```python
from build123d import *

# Parameters (mm, degrees)
SKETCH_1_R          = 62.5
SKETCH_1_R_2        = 45
EXTRUDE_1_DEPTH     = 18
CUT_EXTRUDE_1_DEPTH = 18


with BuildPart() as part:
    # 草图1 → 凸台-拉伸1 (new body)
    with BuildSketch(Plane.XY):
        Circle(SKETCH_1_R)
        Circle(SKETCH_1_R_2, mode=Mode.SUBTRACT)
    extrude(amount=EXTRUDE_1_DEPTH)

    # 草图2 → 切除-旋转1 (revolve, cut)
    with BuildSketch(Plane(origin=(0, 0, 0), x_dir=(1, 0, 0), z_dir=(0, 1, 0)), mode=Mode.PRIVATE) as cut_revolve_1_sk:
        Polygon((62.5, -4), (62.5, 0), (56, 0), align=None)
        Polygon((62.5, -14), (62.5, -18), (56, -18), align=None)
    revolve(cut_revolve_1_sk.sketch.rotate(Axis((0, 0, -32.669833972), (0, 0, 1)), 180), axis=Axis((0, 0, -32.669833972), (0, 0, 1)), mode=Mode.SUBTRACT)

    # 草图3 → 切除-拉伸1 (cut)
    with BuildSketch(Plane(origin=(0, 0, 0), x_dir=(-1, 0, 0), z_dir=(0, 0, -1))):
        with BuildLine():
            Line((-6, 62.211333373), (-6, 57.211333373))
            Line((-6, 57.211333373), (6, 57.211333373))
            Line((6, 57.211333373), (6, 62.211333373))
            ThreePointArc((6, 62.211333373), (0, 62.5), (-6, 62.211333373))
        make_face()
        with BuildLine():
            Line((62.211333373, 6), (57.211333373, 6))
            Line((57.211333373, 6), (57.211333373, -6))
            Line((57.211333373, -6), (62.211333373, -6))
            ThreePointArc((62.211333373, -6), (62.5, 0), (62.211333373, 6))
        make_face()
        with BuildLine():
            Line((6, -62.211333373), (6, -57.211333373))
            Line((6, -57.211333373), (-6, -57.211333373))
            Line((-6, -57.211333373), (-6, -62.211333373))
            ThreePointArc((-6, -62.211333373), (0, -62.5), (6, -62.211333373))
        make_face()
        with BuildLine():
            Line((-62.211333373, -6), (-57.211333373, -6))
            Line((-57.211333373, -6), (-57.211333373, 6))
            Line((-57.211333373, 6), (-62.211333373, 6))
            ThreePointArc((-62.211333373, 6), (-62.5, 0), (-62.211333373, -6))
        make_face()
    extrude(amount=-CUT_EXTRUDE_1_DEPTH, mode=Mode.SUBTRACT)


solid = part.part
```
Can you work these out from the model? Positions are in its coordinate system, mm. A direction names the side the tool comes from. Round coordinates to 2 decimals unless told otherwise and drop trailing zeros. Loops run counter-clockwise (first coordinate to the right, second up) from the corner with the lowest first, then second, coordinate; pieces in that order, holes last. Notation, with made-up numbers: M -8,12.5 L 9,12.5 A35 ccw 9,45.5 Z; hole C 35,37.5 d7. An arc over 180 degrees is marked long. Answer as a JSON object with one key per item and string values. Group by question number.
Q1. We'd pull the mould along Y, two halves only. Please class faces 5 (the flat face through (-57.211, 0, 9)), 6 (the flat face through (60, -6, 9)), 7 (the cylindrical face through (-44.619, -43.766, 8.93)), 8 (the flat face through (6, 60, 9)): +Y half, -Y half, draft (parallel to the pull), parting line (faces both ways), or undercut.
Q2. Imagine slicing it at A-A, the plane y = 0. Please give me the cut outline in (x, z), then the cut area to 3 significant figures.
Q3. Please list where these lines run through material, in increasing order: L1, parallel to Y at x = 0, z = 4.75; L2, parallel to X at y = -38.5, z = 5.75; L3, parallel to Y at x = 13, z = 15.
Q4. On a 3-axis mill with a long thin cutter (end or side, diameter ignored), from which of +Z, -Z, +X, -X, +Y, -Y can I reach the whole of each face in a straight line? I mean faces 1 (the flat face through (60, 6, 9)), 2 (the flat face through (-60, -6, 9)), 3 (the flat face through (-6, 60, 9)), 4 (the flat face through (0, -57.211, 9)). Say none if no direction works.
Q5. Will these pins go through, and if not, where does the flat tip stop? pin 1 (6 mm diameter, centred on y = 2, z = 8.5, fed in from +X); pin 2 (1 mm diameter, centred on x = -3.5, z = 10.5, fed in from +Y); pin 3 (2.5 mm diameter, centred on x = -59, z = 6.5, fed in from +Y).
Q6. Imagine slicing it at B-B, the plane z = 8.75. Please give me the cut outline in (x, y), then the cut area to 3 significant figures.
Findings:
{
 "1": {"face 5": "undercut", "face 6": "undercut", "face 7": "-Y half", "face 8": "draft"},
 "2": {"outline": "M -57.21,0.75 L -56,0 L -45,0 L -45,18 L -56,18 L -57.21,17.25 Z; M 45,0 L 56,0 L 57.21,0.75 L 57.21,17.25 L 56,18 L 45,18 Z", "area": "438 mm2"},
 "3": {"L1": "y = -57.21 to -45, 45 to 57.21", "L2": "x = -49.23 to -23.3, 23.3 to 49.23", "L3": "y = -59.47 to -43.08, 43.08 to 59.47"},
 "4": {"face 1": "+Z, -Z, +X", "face 2": "+Z, -Z, -X", "face 3": "+Z, -Z, +Y", "face 4": "+Z, -Z, -Y"},
 "5": {"pin 1": "stops at x = 57.21", "pin 2": "stops at y = 57.21", "pin 3": "stops at y = 23.9"},
 "6": {"outline": "M -62.21,-6 A62.5 ccw -6,-62.21 L -6,-57.21 L 6,-57.21 L 6,-62.21 A62.5 ccw 62.21,-6 L 57.21,-6 L 57.21,6 L 62.21,6 A62.5 ccw 6,62.21 L 6,57.21 L -6,57.21 L -6,62.21 A62.5 ccw -62.21,6 L -57.21,6 L -57.21,-6 Z; hole C 0,0 d90", "area": "5,660 mm2"}
}
